```python
from build123d import *

# Parameters (mm, degrees)
SKETCH_1_W          = 204
SKETCH_1_H          = 204
EXTRUDE_1_DEPTH     = 10
SKETCH_6_R          = 2.5
CUT_EXTRUDE_1_DEPTH = 3
SKETCH_7_W          = 173
SKETCH_7_H          = 173
EXTRUDE_2_DEPTH     = 10


with BuildPart() as part:
    # 草图1 → 凸台-拉伸1 (new body)
    with BuildSketch(Plane.XY):
        Rectangle(SKETCH_1_W, SKETCH_1_H)
    extrude(amount=EXTRUDE_1_DEPTH)

    # 切除-扫描2: sweep along a path in 草图2
    with BuildLine(Plane.XY.offset(10)) as sweep_2_path:
        Line((-80, -80), (80, -80))
        Line((80, -80), (80, 80))
        Line((80, 80), (-80, 80))
        Line((-80, 80), (-80, -80))
    # 草图3 → 切除-扫描2 (sweep, cut)
    with BuildSketch(Plane(origin=(0, 0, 0), x_dir=(1, 0, 0), z_dir=(0, 1, 0))):
        Polygon((-88.948256764, -10), (-88.948256764, -8.70522639), (-82.270562222, -10), align=None)
    sweep(path=sweep_2_path.line, transition=Transition.RIGHT, mode=Mode.SUBTRACT)

    # 切除-扫描3: sweep along a path in 草图4
    with BuildLine(Plane.XY.offset(10)) as sweep_3_path:
        Line((-70, -70), (70, -70))
        Line((70, -70), (70, 70))
        Line((70, 70), (-70, 70))
        Line((-70, 70), (-70, -70))
    # 草图5 → 切除-扫描3 (sweep, cut)
    with BuildSketch(Plane(origin=(0, 0, 0), x_dir=(1, 0, 0), z_dir=(0, 1, 0))):
        Polygon((-70.048782141, -10), (-70.048782141, -6.864221928), (-59.608863027, -10), align=None)
    sweep(path=sweep_3_path.line, transition=Transition.RIGHT, mode=Mode.SUBTRACT)

    # 草图6 → 切除-拉伸1 (cut)
    with BuildSketch(Plane(origin=(0, 0, 0), x_dir=(-1, 0, 0), z_dir=(0, 0, -1))):
        with Locations((-92, 92)):
            Circle(SKETCH_6_R)
        with Locations((92, 92)):
            Circle(SKETCH_6_R)
        with Locations((-92, -92)):
            Circle(SKETCH_6_R)
        with Locations((92, -92)):
            Circle(SKETCH_6_R)
    extrude(amount=-CUT_EXTRUDE_1_DEPTH, mode=Mode.SUBTRACT)

    # 草图7 → 凸台-拉伸2 (add)
    with BuildSketch(Plane(origin=(0, 0, 0), x_dir=(-1, 0, 0), z_dir=(0, 0, -1))):
        Rectangle(SKETCH_7_W, SKETCH_7_H)
    extrude(amount=EXTRUDE_2_DEPTH)


solid = part.part
```
For this review, take the finished solid that the model builds, in its own axes (mm). A direction names the side the tool comes from. Give positions to 0.01 mm unless a question says otherwise; leave off trailing zeros. Write each loop counter-clockwise with the first axis right and the second up, starting at its lowest first coordinate (ties: lowest second). Pieces come first, ordered by that corner, then holes. Notation, with made-up numbers: M 15.5,69.25 L 52.5,69.25 A27 ccw 52.5,86.25 Z; hole C -39,17 d11. An arc over 180 degrees is marked long. One line per item, written item: value.
1) Take a section at C-C, the plane z = -7.5. Write out the cut boundary in (x, y), then the cut area to 3 significant figures.
Results are:
outline: M -86.5,-86.5 L 86.5,-86.5 L 86.5,86.5 L -86.5,86.5 Z
area: 29,900 mm²
2) For P1, Ø1.5, axis at x = 91.5, y = 91, coming from the -Z side; P2, Ø5.5, axis at x = -92.5, y = -93, coming from the -Z side; P3, Ø5, axis at x = -37.5, z = -3.5, coming from the -Y side, all flat-tipped, find the tip position at first contact; note any pin that passes through.
Results are:
P1: stops at z = 3
P2: stops at z = 0
P3: stops at y = -86.5
3) For line 1 (Y direction, x = 92, z = 2.15); line 2 (Y direction, x = -21, z = -9), list the stretches that pass through material, from the lowest coordinate up. Write a range as from..to.
Results are:
line 1: y = -102..-94.5, -89.5..89.5, 94.5..102
line 2: y = -86.5..86.5
4) Take a section at A-A, the plane y = -1. Write out the cut boundary in (x, z).
Results are:
outline: M -102,0 L -86.5,0 L -86.5,-10 L 86.5,-10 L 86.5,0 L 102,0 L 102,10 L 88.95,10 L 88.95,8.71 L 82.27,10 L 70.05,10 L 70.05,6.86 L 59.61,10 L -59.61,10 L -70.05,6.86 L -70.05,10 L -82.27,10 L -88.95,8.71 L -88.95,10 L -102,10 Z
5) Take a section at B-B, the plane x = -92. Write out the cut boundary in (y, z).
Results are:
outline: M -102,0 L -94.5,0 L -94.5,3 L -89.5,3 L -89.5,0 L 89.5,0 L 89.5,3 L 94.5,3 L 94.5,0 L 102,0 L 102,10 L -102,10 Z
6) The part is to be moulded in two halves that separate along Y. For faces 1 (the flat face through (1, 86.5, -5)), 2 (the cylindrical face through (92.33, -89.52, 1.48)), 3 (the flat face through (1, -86.5, -5)), 4 (the flat face through (102, -1, 5)), say which applies: +Y half, -Y half, draft (parallel to the pull), parting line (faces both ways), or undercut.
Results are:
face 1: +Y half
face 2: undercut
face 3: -Y half
face 4: draft
7) For faces 5 (the flat face through (0.981, -64.756, 8.454)), 6 (the cylindrical face through (92.33, 94.48, 1.48)), 7 (the flat face through (-86.5, -1, -5)), list the 3-axis set-ups (+Z, -Z, +X, -X, +Y, -Y) from which the entire face can be reached by the end or side of a thin tool; tool diameter is ignored.
Results are:
face 5: +Z
face 6: -Z
face 7: -Z, -X, +Y, -Y
